Can you work these out from the drawing? Everything is in mm from the part's minimum corner. Give positions to 0.01 mm unless a question says otherwise; leave off trailing zeros. Write each loop counter-clockwise with the first axis right and the second up, starting at its lowest first coordinate (ties: lowest second). Pieces come first, ordered by that corner, then holes. Notation, with made-up numbers: (-15.5, 53) - (25.5, 53) arc R28 ccw to (25.5, 76) - close; hole circle Ø4 at (26, 31). An arc over 180 degrees is marked (long way). Answer in a Markdown table with one row per item.
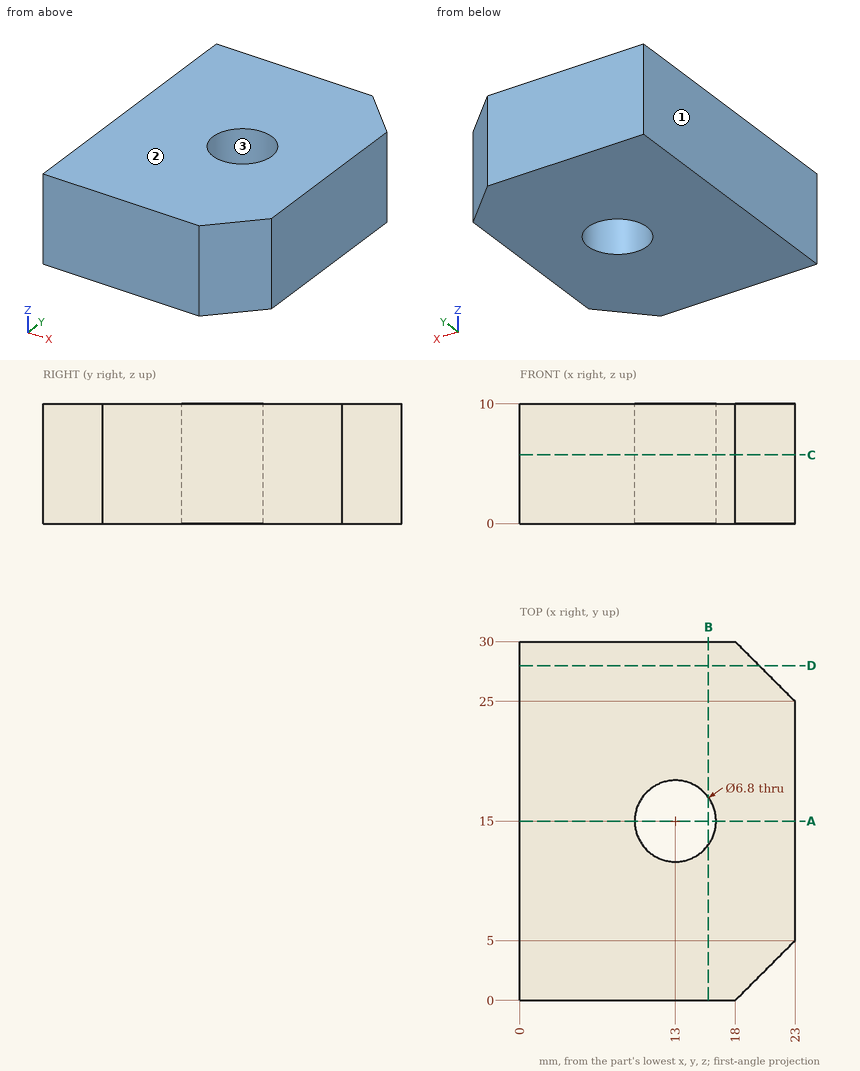
1) Imagine slicing it at B-B (x = 15.75). List the corners of the cut face in (y, z) for me, then the cut area to 3 significant figures.
Check values:
| item | result |
|---|---|
| outline | (0, 0) - (13, 0) - (13, 10) - (0, 10) - close; (17, 0) - (30, 0) - (30, 10) - (17, 10) - close |
| area | 260 mm2 |
2) If I drill on line 1 (Y direction, x = 13, z = 3.5); line 2 (X direction, y = 18, z = 3.5); line 3 (X direction, y = 16.75, z = 9), over which ranges is the centre line in solid material (lowest first)?
Check values:
| item | result |
|---|---|
| line 1 | y = 0 to 11.6, 18.4 to 30 |
| line 2 | x = 0 to 11.4, 14.6 to 23 |
| line 3 | x = 0 to 10.08, 15.92 to 23 |
3) Will this pin go through, and if not, where does the flat tip stop? P1, Ø3, axis at x = 7.5, z = 3, coming from the -Y side.
Check values:
| item | result |
|---|---|
| P1 | stops at y = 0 |
4) Imagine slicing it at C-C (z = 5.75). List the corners of the cut face in (x, y) for me, then the cut area to 3 significant figures.
Check values:
| item | result |
|---|---|
| outline | (0, 0) - (18, 0) - (23, 5) - (23, 25) - (18, 30) - (0, 30) - close; hole circle Ø6.8 at (13, 15) |
| area | 629 mm2 |
5) Imagine slicing it at A-A (y = 15). List the corners of the cut face in (x, z) for me, then the cut area to 3 significant figures.
Check values:
| item | result |
|---|---|
| outline | (0, 0) - (9.6, 0) - (9.6, 10) - (0, 10) - close; (16.4, 0) - (23, 0) - (23, 10) - (16.4, 10) - close |
| area | 162 mm2 |
6) We'd pull the mould along X, two halves only. Please class the marked faces 1, 2 and 3: +X half, -X half, draft (parallel to the pull), parting line (faces both ways), or undercut.
Check values:
| item | result |
|---|---|
| face 1 | -X half |
| face 2 | draft |
| face 3 | undercut |
7) Imagine slicing it at D-D (y = 28). List the corners of the cut face in (x, z) for me.
Check values:
| item | result |
|---|---|
| outline | (0, 0) - (20, 0) - (20, 10) - (0, 10) - close |
